Check sheet for the modelled part. Datum: model origin and axes. Units: mm. A direction names the side the tool comes from. Round coordinates to 2 decimals unless told otherwise and drop trailing zeros. Write each loop counter-clockwise with the first axis right and the second up, starting at its lowest first coordinate (ties: lowest second). Pieces come first, ordered by that corner, then holes. Notation, with made-up numbers: M 19.5,12 L 32.5,12 A4 cw 32.5,16 Z; hole C -11,2 d1. An arc over 180 degrees is marked long. One line per item, written item: value.
from build123d import *

# Parameters (mm, degrees)
SKETCH1_W                          = 75
SKETCH1_H                          = 144
BOSS_EXTRUDE1_DEPTH                = 6
SKETCH4_W                          = 15
SKETCH4_H                          = 114
CUT_EXTRUDE1_DEPTH                 = 83.0624762
F_6_6_6_6_DIAMETER_HOLE1_D         = 6.6
BLIND_PIN_HOLE1_SIZE_MM_AT_2_COUNT = 2
BLIND_PIN_HOLE1_SIZE_MM_AT_2_PITCH = 30
CHAMFER1_SIZE                      = 1


with BuildPart() as part:
    # Sketch1 → Boss-Extrude1 (new, symmetric)
    with BuildSketch(Plane.XY):
        Rectangle(SKETCH1_W, SKETCH1_H)
    extrude(amount=BOSS_EXTRUDE1_DEPTH, both=True)

    # Sketch4 → Cut-Extrude1 (cut, through all)
    with BuildSketch(Plane.XY.offset(6)):
        with Locations((-30, 0)):
            Rectangle(SKETCH4_W, SKETCH4_H)
    cut_extrude1 = extrude(amount=-CUT_EXTRUDE1_DEPTH, mode=Mode.SUBTRACT)

    # Mirror1: Cut-Extrude1 across plane
    add(cut_extrude1.mirror(Plane(origin=(0, 0, 0), x_dir=(0, 0, 1), z_dir=(1, 0, 0))), mode=Mode.SUBTRACT)

    # Ø6.6 (6.6) Diameter Hole1 (through all)
    with Locations(Plane(origin=(0, -72, 0), x_dir=(-1, 0, 0), z_dir=(0, -1, 0))):
        with Locations((-30, 0), (30, 0)):
            Hole(F_6_6_6_6_DIAMETER_HOLE1_D / 2)

    # Sketch8 → Blind Pin Hole1 (size mm) (revolve, cut)
    with BuildSketch(Plane(origin=(15, -72, 0), x_dir=(0, 0, -1), z_dir=(1, 0, 0))):
        Polygon((0, 0), (0, 12.502151548), (2.5, 11), (2.5, 0), align=None)
    blind_pin_hole1_size_mm = revolve(axis=Axis((15, -78.35, 0), (0, 1, 0)), mode=Mode.SUBTRACT)

    # Blind Pin Hole1 (size mm) at 2: Blind Pin Hole1 (size mm) ×2
    with Locations(*[(-i * BLIND_PIN_HOLE1_SIZE_MM_AT_2_PITCH, 0, 0) for i in range(1, BLIND_PIN_HOLE1_SIZE_MM_AT_2_COUNT)]):
        add(blind_pin_hole1_size_mm, mode=Mode.SUBTRACT)

    # Mirror2: Blind Pin Hole1 (size mm) across plane
    add(blind_pin_hole1_size_mm.mirror(Plane.ZX), mode=Mode.SUBTRACT)

    # Mirror2 copy 1 sketch → Mirror2 copy 1 (revolve, cut)
    with BuildSketch(Plane(origin=(-15, 72, 0), x_dir=(0, 0, -1), z_dir=(1, 0, 0))):
        Polygon((0, 0), (0, -12.502151548), (2.5, -11), (2.5, 0), align=None)
    revolve(axis=Axis((-15, 78.35, 0), (0, 1, 0)), mode=Mode.SUBTRACT)

    # Chamfer1
    chamfer1_edges = [part.edges().sort_by_distance(p)[0] for p in [
        (-37.5, 64.5, 6),
        (-37.5, -64.5, -6),
        (-37.5, -64.5, 6),
        (37.5, 64.5, -6),
        (37.5, 64.5, 6),
        (37.5, -64.5, 6),
        (-37.5, 64.5, -6),
        (37.5, -64.5, -6),
    ]]
    chamfer(chamfer1_edges, length=CHAMFER1_SIZE)


solid = part.part
Q1. Sectioned sample at B-B on y = 42. Enter the section's corners in (x, z).
Completed:
outline: M -22.5,-6 L 22.5,-6 L 22.5,6 L -22.5,6 Z
Q2. Draft check along Z on faces 1 (the flat face through (-22.5, -1, 0)), 2 (the conical face through (-15.37, -59.76, -0.23)), 3 (the flat face through (-1, 1, -6)). Enter one of: pulls with the +Z half, pulls with the -Z half, needs draft (parallel to the pull), parting line crosses it, or undercut.
Completed:
face 1: needs draft
face 2: undercut
face 3: pulls with the -Z half
Q3. Access from +Z, -Z, +X, -X, +Y, -Y to the whole of each face (thin tool, end or side, straight path). Record for faces 4 (the cylindrical face through (17.44, 66.58, 0.54)), 5 (the cylindrical face through (-12.56, -66.58, 0.54)), 6 (the flat face through (22.5, -1, 0)), 7 (the flat face through (-33.4, -57, 1.4)).
Completed:
face 4: +Y
face 5: -Y
face 6: +Z, -Z, +X
face 7: +Z, -Z, -X
Q4. Scan lines: line 1 (Y direction, x = 24, z = -1.75); line 2 (Z direction, x = 30, y = 65.5); line 3 (Z direction, x = -15, y = 68.25). Record each from-to range of solid material in increasing order. Write a range as [from, to].
Completed:
line 1: [-72, -57], [57, 72]
line 2: [-6, -3.3], [3.3, 6]
line 3: [-6, -2.5], [2.5, 6]
Q5. Sectioned sample at A-A on x = -30. Enter the section's corners in (y, z), and give its area (3 significant figures).
Completed:
outline: M -72,-6 L -57,-6 L -57,-3.3 L -72,-3.3 Z; M -72,3.3 L -57,3.3 L -57,6 L -72,6 Z; M 57,-6 L 72,-6 L 72,-3.3 L 57,-3.3 Z; M 57,3.3 L 72,3.3 L 72,6 L 57,6 Z
area: 162 mm^2
Q6. Depth check by flat-ended pin: P1, Ø5.5, axis at x = 30, z = 0, coming from the +Y side; P2, Ø4.5, axis at x = 15, z = 0, coming from the -Y side; P3, Ø1.5, axis at y = 37, z = -1, coming from the -X side; P4, Ø4.5, axis at x = -15, z = 0, coming from the +Y side. Enter the tip coordinate at first touch or a pass-through.
Completed:
P1: through
P2: y = -60.85
P3: x = -22.5
P4: y = 60.85
